Verification items for the finished model (mm, model axes). A direction names the side the tool comes from. Round coordinates to 2 decimals unless told otherwise and drop trailing zeros. Order: outer loops, then holes, each group sorted by start corner. A loop starts at its lowest first (then second) coordinate and runs counter-clockwise, first axis right, second up. Notation, with made-up numbers: (-8.5, -18.5) -> (39.5, -18.5) arc R23 ccw to (39.5, -8.5) -> close; hole circle Ø11 at (20.5, 89). An arc over 180 degrees is marked (long way). Return JSON: item names as keys, results as strings. Group by question number.
1) Depth check by flat-ended pin: pin 1 (11 mm diameter, centred on x = 9, z = 16, fed in from -Y); pin 2 (1.5 mm diameter, centred on x = -2, z = 8.5, fed in from +Y); pin 3 (5 mm diameter, centred on x = 8.5, z = -16.5, fed in from -Y). Enter the tip coordinate at first touch or a pass-through.
2) Draft check along X on faces 4 (the conical face through (-18.1, -0.1, -10.7)), 5 (the cylindrical face through (-0.845, 0.056, 8.979)), 6 (the flat face through (0, 0, 21)). Enter one of: pulls with the +X half, pulls with the -X half, needs draft (parallel to the pull), parting line crosses it, or undercut.
3) Section check B-B on x = 7. Enter the section's corners in (y, z), plus the area to 3 significant figures.
4) Scan lines: L1, parallel to Z at x = 7, y = 2.8; L2, parallel to Z at x = 7, y = -0.9; L3, parallel to Y at x = -21, z = 11. Record each from-to range of solid material in increasing order.
5) Section check A-A on z = -15. Enter the section's corners in (x, y).
6) Tool access check on faces 1 (the cylindrical face through (-23.879, -0.632, -12.524)), 2 (the cylindrical face through (4.693, -1.338, -10.564)), 3 (the cylindrical face through (-17.25, 0.06, 8.45)). Record the directions out of +Z, -Z, +X, -X, +Y, -Y that give a thin tool (end or side, any length) a straight path to the whole face; none if there is none.
7) Section check C-C on y = 2.25. Enter the section's corners in (x, z), plus the area to 3 significant figures.
8) Section check D-D on x = -16. Enter the section's corners in (y, z), plus the area to 3 significant figures.
```python
from build123d import *

# Parameters (mm, degrees)
SKETCH_1_W                   = 58
SKETCH_1_H                   = 42
EXTRUDE_1_DEPTH              = 4
HOLE_WIZARD_M5_1_D           = 5.5
HOLE_WIZARD_M5_1_CBORE_D     = 10
HOLE_WIZARD_M5_1_CBORE_DEPTH = 5.4
HOLE_WIZARD_M4_1_D           = 3.3
HOLE_WIZARD_M4_1_DEPTH       = 10.1
HOLE_WIZARD_M4_1_TIP         = 0.991420021
HOLE_WIZARD_M3_1_D           = 2.5


with BuildPart() as part:
    # 草图1 → 凸台-拉伸1 (new, symmetric)
    with BuildSketch(Plane(origin=(0, 0, 0), x_dir=(1, 0, 0), z_dir=(0, 1, 0))):
        Rectangle(SKETCH_1_W, SKETCH_1_H)
    extrude(amount=EXTRUDE_1_DEPTH, both=True)

    # M5 六角凹头螺钉的柱形沉头孔1 (through all)
    with Locations(Plane(origin=(0, -4, 0), x_dir=(-1, 0, 0), z_dir=(0, -1, 0))):
        with Locations((-7, 15), (-7, -15)):
            CounterBoreHole(HOLE_WIZARD_M5_1_D / 2, HOLE_WIZARD_M5_1_CBORE_D / 2, HOLE_WIZARD_M5_1_CBORE_DEPTH)

    # M4 螺纹孔1
    with Locations(Plane.ZY.offset(29)):
        with Locations((-11, 0), (11, 0)):
            Hole(HOLE_WIZARD_M4_1_D / 2, depth=HOLE_WIZARD_M4_1_DEPTH)
            with Locations((0, 0, -(HOLE_WIZARD_M4_1_DEPTH + HOLE_WIZARD_M4_1_TIP / 2))):  # 118° drill point
                Cone(0, HOLE_WIZARD_M4_1_D / 2, HOLE_WIZARD_M4_1_TIP, mode=Mode.SUBTRACT)

    # M3 螺纹孔1 (through all)
    with Locations(Plane(origin=(0, -4, 0), x_dir=(-1, 0, 0), z_dir=(0, -1, 0))):
        with Locations((16, -8.5), (2, -8.5)):
            Hole(HOLE_WIZARD_M3_1_D / 2)


solid = part.part
```
Check result:
{
 "1": {"pin 1": "y = -4", "pin 2": "through", "pin 3": "y = 1.4"},
 "2": {"face 4": "pulls with the -X half", "face 5": "undercut", "face 6": "needs draft"},
 "3": {"outline": "(-4, -21) -> (4, -21) -> (4, -17.75) -> (1.4, -17.75) -> (1.4, -20) -> (-4, -20) -> close; (-4, -10) -> (1.4, -10) -> (1.4, -12.25) -> (4, -12.25) -> (4, 12.25) -> (1.4, 12.25) -> (1.4, 10) -> (-4, 10) -> close; (-4, 20) -> (1.4, 20) -> (1.4, 17.75) -> (4, 17.75) -> (4, 21) -> (-4, 21) -> close", "area": "199 mm^2"},
 "4": {"L1": "-21 to -17.75, -12.25 to 12.25, 17.75 to 21", "L2": "-21 to -20, -10 to 10, 20 to 21", "L3": "-4 to -1.65, 1.65 to 4"},
 "5": {"outline": "(-29, -4) -> (2, -4) -> (2, 1.4) -> (4.25, 1.4) -> (4.25, 4) -> (-29, 4) -> close; (9.75, 1.4) -> (12, 1.4) -> (12, -4) -> (29, -4) -> (29, 4) -> (9.75, 4) -> close"},
 "6": {"face 1": "-X", "face 2": "-Y", "face 3": "+Y, -Y"},
 "7": {"outline": "(-29, -21) -> (29, -21) -> (29, 21) -> (-29, 21) -> close; hole circle Ø2.5 at (-16, 8.5); hole circle Ø2.5 at (-2, 8.5); hole circle Ø5.5 at (7, -15); hole circle Ø5.5 at (7, 15)", "area": "2,380 mm^2"},
 "8": {"outline": "(-4, -21) -> (4, -21) -> (4, 7.25) -> (-4, 7.25) -> close; (-4, 9.75) -> (4, 9.75) -> (4, 21) -> (-4, 21) -> close", "area": "316 mm^2"}
}
